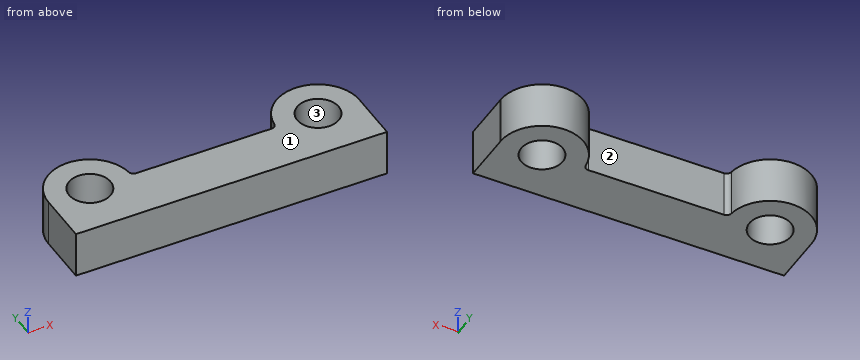
from build123d import *

# Parameters (mm, degrees)
SKETCH1_R           = 40
BOSS_EXTRUDE2_DEPTH = 90


with BuildPart() as part:
    # Sketch1 → Boss-Extrude2 (new body)
    with BuildSketch(Plane.XY):
        with BuildLine():
            ThreePointArc((-140.4953608, 8.888888889), (-224.451340472, 79.876063799), (-300, 0))
            Line((-300, 0), (-300, -100))
            Line((-300, -100), (300, -100))
            Line((300, -100), (299.972882257, -2.08281146))
            Line((299.972882257, -2.08281146), (299.971716338, 2.127107427))
            ThreePointArc((299.971716338, 2.127107427), (223.388947093, 79.928186753), (140.4953608, 8.888888889))
            ThreePointArc((140.4953608, 8.888888889), (137.223947567, 2.546440075), (130.5572809, 0))
            Line((130.5572809, 0), (-130.5572809, 0))
            ThreePointArc((-130.5572809, 0), (-137.223947567, 2.546440075), (-140.4953608, 8.888888889))
        make_face()
        with Locations(Location((-220, 0, 0), (0, 0, 180))):
            Circle(SKETCH1_R, mode=Mode.SUBTRACT)
        with Locations(Location((220, 0, 0), (0, 0, 180))):
            Circle(SKETCH1_R, mode=Mode.SUBTRACT)
    extrude(amount=BOSS_EXTRUDE2_DEPTH)


solid = part.part
Geometry: final body of the model. Coordinates: model frame, mm. Face numbers are marked on the shaded views. Coordinates: 2 decimals unless noted, no trailing zeros. Write each loop counter-clockwise with the first axis right and the second up, starting at its lowest first coordinate (ties: lowest second). Pieces come first, ordered by that corner, then holes. Notation, with made-up numbers: (-4, 85) - (18, 85) arc R19 ccw to (18, 94) - close; hole circle Ø6 at (51, 81.25). An arc over 180 degrees is marked (long way). Return JSON: item names as keys, results as strings.
Item 1: Section query A-A (z = 45). Output: boundary loops of the cut face in (x, y).
Completed:
{"outline": "(-300, -100) - (300, -100) - (299.97, 2.13) arc R80 ccw to (140.5, 8.89) arc R10 cw to (130.56, 0) - (-130.56, 0) arc R10 cw to (-140.5, 8.89) arc R80 ccw to (-300, 0) - close; hole circle Ø80 at (-220, 0); hole circle Ø80 at (220, 0)"}
Item 2: Section query C-C (y = 53.5). Output: boundary loops of the cut face in (x, z), and give its area (3 significant figures).
Completed:
{"outline": "(-279.48, 0) - (-160.52, 0) - (-160.52, 90) - (-279.48, 90) - close; (160.52, 0) - (279.48, 0) - (279.48, 90) - (160.52, 90) - close", "area": "21,400 mm2"}
Item 3: Pin query (flat end, axial travel): pin 1 Ø6 at (x, z) = (-54.5, 73) entering from +Y; pin 2 Ø4.5 at (y, z) = (1, 37.5) entering from +X; pin 3 Ø12 at (y, z) = (48.5, 75) entering from -X. Return the tip coordinate at first contact, or that it passes through.
Completed:
{"pin 1": "stops at y = 0", "pin 2": "stops at x = 299.97", "pin 3": "stops at x = -287.78"}
Item 4: Section query D-D (y = -20.5). Output: boundary loops of the cut face in (x, z).
Completed:
{"outline": "(-300, 0) - (-254.35, 0) - (-254.35, 90) - (-300, 90) - close; (-185.65, 0) - (185.65, 0) - (185.65, 90) - (-185.65, 90) - close; (254.35, 0) - (299.98, 0) - (299.98, 90) - (254.35, 90) - close"}
Item 5: Line query: L1, parallel to Y at x = 220, z = 32.5; L2, parallel to X at y = -10, z = 37.5; L3, parallel to Y at x = -93.5, z = 48.5. Output: solid intervals per line, ascending.
Completed:
{"L1": "y = -100 to -40, 40 to 80", "L2": "x = -300 to -258.73, -181.27 to 181.27, 258.73 to 299.98", "L3": "y = -100 to 0"}
Item 6: Pull-direction query (Y, two-part tool) for the marked faces 1, 2 and 3; classes: +Y half, -Y half, draft (parallel to the pull), parting line (faces both ways), or undercut.
Completed:
{"face 1": "draft", "face 2": "+Y half", "face 3": "undercut"}
Item 7: Section query B-B (x = -186). Output: boundary loops of the cut face in (y, z), and give its area (3 significant figures).
Completed:
{"outline": "(-100, 0) - (-21.07, 0) - (-21.07, 90) - (-100, 90) - close; (21.07, 0) - (72.42, 0) - (72.42, 90) - (21.07, 90) - close", "area": "11,700 mm2"}
